from build123d import *

# Parameters (mm, degrees)
SKETCH1_R           = 93
BOSS_EXTRUDE1_DEPTH = 20


with BuildPart() as part:
    # Sketch1 → Boss-Extrude1 (new body)
    with BuildSketch(Plane.XY):
        with BuildLine():
            Line((-99, 0), (99, 0))
            Line((99, 0), (99, 20))
            Line((99, 20), (124.5, 20))
            Line((124.5, 20), (136.5, 32))
            Line((136.5, 32), (136.5, 180.6))
            ThreePointArc((136.5, 180.6), (131.613179244, 195.447896171), (118.863198343, 204.491071767))
            Line((118.863198343, 204.491071767), (10.30847768, 237.947500473))
            ThreePointArc((10.30847768, 237.947500473), (0, 239.5), (-10.30847768, 237.947500473))
            Line((-10.30847768, 237.947500473), (-118.863198343, 204.491071767))
            ThreePointArc((-118.863198343, 204.491071767), (-131.613179244, 195.447896171), (-136.5, 180.6))
            Line((-136.5, 180.6), (-136.5, 32))
            Line((-136.5, 32), (-124.5, 20))
            Line((-124.5, 20), (-99, 20))
            Line((-99, 20), (-99, 0))
        make_face()
        with Locations((0, 116)):
            Circle(SKETCH1_R, mode=Mode.SUBTRACT)
    extrude(amount=BOSS_EXTRUDE1_DEPTH)


solid = part.part
Read the model definition and answer for the solid it produces. Units are mm, in the model's axes. A direction names the side the tool comes from. Round coordinates to 2 decimals unless told otherwise and drop trailing zeros. Write each loop counter-clockwise with the first axis right and the second up, starting at its lowest first coordinate (ties: lowest second). Pieces come first, ordered by that corner, then holes.
1. Which of the six approach directions +Z, -Z, +X, -X, +Y, -Y give full straight-line access (tool end or side, diameter ignored) to faces 1 (the face through (99, 10, 10)), 2 (the face through (-112, 20, 10)), 3 (the face through (136.5, 105, 10))?
2. The part is cut by section D-D, the plane x = 96. Determine the outline of the cut face in (y, z), then the cut area to 3 significant figures.
3. The part is cut by section B-B, the plane x = 0. Determine the outline of the cut face in (y, z), then the cut area to 3 significant figures.
4. Straight lines are drawn through the part: L1, parallel to Y at x = 0, z = 5.25; L2, parallel to X at y = 38, z = 2.5; L3, parallel to Y at x = -49, z = 16.75. For each, find the intervals that lie inside material, in ascending order.
5. Determine the mould class of faces 4 (the face through (-99, 10, 10)), 5 (the face through (131.745, 195.268, 9.86)), 6 (the face through (-20.16, 25.21, 9.86)) for opening direction Y: pulls with the +Y half, pulls with the -Y half, needs draft (parallel to the pull), parting line crosses it, or undercut.
6. Given pin 1 Ø2 at (y, z) = (186, 11.5) entering from +X; pin 2 Ø6 at (x, z) = (-109.5, 14) entering from -Y, each flat-ended and moving along its own axis, determine where each tip first touches the part or whether it passes through.
7. The part is cut by section A-A, the plane z = 3.25. Determine the outline of the cut face in (x, y).
8. The part is cut by section C-C, the plane y = 116. Determine the outline of the cut face in (x, z).
Values:
1. face 1: +Z, -Z, +X, -Y
1. face 2: +Z, -Z, -X, -Y
1. face 3: +Z, -Z, +X, +Y, -Y
2. outline: (0, 0) - (211.54, 0) - (211.54, 20) - (0, 20) - close
2. area: 4,230 mm2
3. outline: (0, 0) - (23, 0) - (23, 20) - (0, 20) - close; (209, 0) - (239.5, 0) - (239.5, 20) - (209, 20) - close
3. area: 1,070 mm2
4. L1: y = 0 to 23, 209 to 239.5
4. L2: x = -136.5 to -50.65, 50.65 to 136.5
4. L3: y = 0 to 36.96, 195.04 to 226.02
5. face 4: needs draft
5. face 5: pulls with the +Y half
5. face 6: undercut
6. pin 1: stops at x = 136.11
6. pin 2: stops at y = 20
7. outline: (-136.5, 32) - (-124.5, 20) - (-99, 20) - (-99, 0) - (99, 0) - (99, 20) - (124.5, 20) - (136.5, 32) - (136.5, 180.6) arc R25 ccw to (118.86, 204.49) - (10.31, 237.95) arc R35 ccw to (-10.31, 237.95) - (-118.86, 204.49) arc R25 ccw to (-136.5, 180.6) - close; hole circle Ø186 at (0, 116)
8. outline: (-136.5, 0) - (-93, 0) - (-93, 20) - (-136.5, 20) - close; (93, 0) - (136.5, 0) - (136.5, 20) - (93, 20) - close
